Here's how the part is built. I have some questions about the finished solid (model axes, mm). A direction names the side the tool comes from. Give positions to 0.01 mm unless a question says otherwise; leave off trailing zeros. Loops run counter-clockwise (first coordinate to the right, second up) from the corner with the lowest first, then second, coordinate; pieces in that order, holes last.
Q1. Thinking about a two-plate mould opening in X: for faces 3 (the face through (0, 20, 1)), 4 (the face through (20, 0, 1)), 5 (the face through (17, 0, 1)), 6 (the face through (0, 17, 1)), which applies, pulls with the +X half, pulls with the -X half, needs draft (parallel to the pull), parting line crosses it, or undercut?
Q2. Suppose I cut it at A-A (x = -4.5). List the corners of the cut face in (y, z) for me, and give its area (3 significant figures).
Q3. Suppose I cut it at C-C (z = -14.5). List the corners of the cut face in (x, y) for me, and give its area (3 significant figures).
Q4. I need wall thicknesses on probe 1 along Y at (x, z) = (9, -40). Which ranges of the line are inside material? Lowest first, please.
Q5. For faces 1 (the face through (-20, 0, 1)), 2 (the face through (0, -17, 1)), which set-ups out of +Z, -Z, +X, -X, +Y, -Y let a thin tool reach every point of the face, with its end or its side?
Q6. I'm going to push a flat-ended pin straight in: P1, Ø3, axis at x = 7.5, y = -14.5, coming from the +Z side. Where does the tip first touch, or does it pass through?
```python
from build123d import *

# Parameters (mm, degrees)
SKETCH_1_W      = 40
SKETCH_1_H      = 40
SKETCH_1_W_2    = 34
SKETCH_1_H_2    = 34
EXTRUDE_1_DEPTH = 48.5


with BuildPart() as part:
    # 草图1 → 凸台-拉伸1 (new, symmetric)
    with BuildSketch(Plane.XY):
        Rectangle(SKETCH_1_W, SKETCH_1_H)
        Rectangle(SKETCH_1_W_2, SKETCH_1_H_2, mode=Mode.SUBTRACT)
    extrude(amount=EXTRUDE_1_DEPTH, both=True)


solid = part.part
```
Solutions:
1. face 3: needs draft
1. face 4: pulls with the +X half
1. face 5: undercut
1. face 6: undercut
2. outline: (-20, -48.5) - (-17, -48.5) - (-17, 48.5) - (-20, 48.5) - close; (17, -48.5) - (20, -48.5) - (20, 48.5) - (17, 48.5) - close
2. area: 582 mm2
3. outline: (-20, -20) - (20, -20) - (20, 20) - (-20, 20) - close; hole (-17, -17) - (17, -17) - (17, 17) - (-17, 17) - close
3. area: 444 mm2
4. probe 1: y = -20 to -17, 17 to 20
5. face 1: +Z, -Z, -X, +Y, -Y
5. face 2: +Z, -Z
6. P1: passes through
